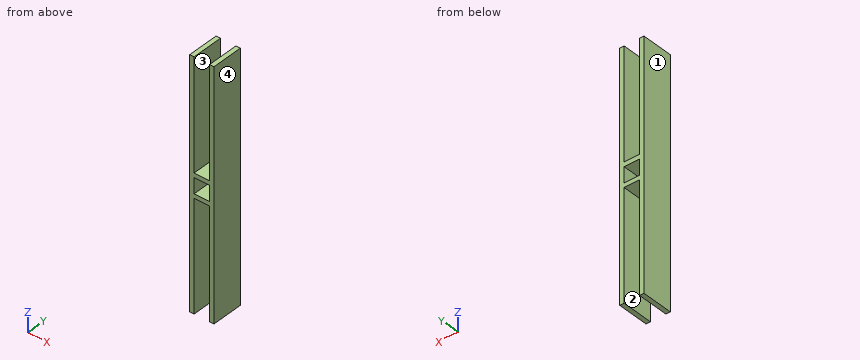
```python
from build123d import *

# Parameters (mm, degrees)
SKETCH1_W           = 10
SKETCH1_H           = 71
BOSS_EXTRUDE1_DEPTH = 556
SKETCH2_W           = 10
SKETCH2_H           = 71
BOSS_EXTRUDE2_DEPTH = 35
SKETCH3_W           = 10
SKETCH3_H           = 556
BOSS_EXTRUDE3_DEPTH = 71


with BuildPart() as part:
    # Sketch1 → Boss-Extrude1 (new body)
    with BuildSketch(Plane.XY):
        Rectangle(SKETCH1_W, SKETCH1_H)
    extrude(amount=BOSS_EXTRUDE1_DEPTH)

    # Sketch2 → Boss-Extrude2 (add)
    with BuildSketch(Plane(origin=(5, 0, 0), x_dir=(0, 0, -1), z_dir=(1, 0, 0))):
        with Locations((-300, 0)):
            Rectangle(SKETCH2_W, SKETCH2_H)
        with Locations((-255, 0)):
            Rectangle(SKETCH2_W, SKETCH2_H)
    extrude(amount=BOSS_EXTRUDE2_DEPTH)

    # Sketch3 → Boss-Extrude3 (add)
    with BuildSketch(Plane(origin=(0, 35.5, 0), x_dir=(1, 0, 0), z_dir=(0, 1, 0))):
        with Locations((45, -278)):
            Rectangle(SKETCH3_W, SKETCH3_H)
    extrude(amount=-BOSS_EXTRUDE3_DEPTH)


solid = part.part
```
The listing builds one solid part. Answer for the finished solid, in the listing's coordinates (mm). Face numbers are marked on the shaded views. Give positions to 0.01 mm unless a question says otherwise; leave off trailing zeros. Loops run counter-clockwise (first coordinate to the right, second up) from the corner with the lowest first, then second, coordinate; pieces in that order, holes last. Notation, with made-up numbers: (36.25, 73) - (44.25, 73) arc R25 ccw to (44.25, 86) - close; hole circle Ø1 at (31, 25). An arc over 180 degrees is marked (long way). Answer as CSV lines item,"result". Start each with the question number.
Item 1: Find the intervals of material crossed by line 1 (Z direction, x = 9, y = 13); line 2 (X direction, y = 23.5, z = 91.5), in increasing order. Write a range as from..to.
Item 2: This flat-tipped pin is pushed along its axis until it touches: pin 1 (4 mm diameter, centred on x = 39, z = 318.5, fed in from +Y). Where does it stop, or does it pass through?
Item 3: A cutting plane is placed at C-C on y = -27. Determine the outline of the cut face in (x, z), then the cut area to 3 significant figures.
Item 4: The mould has two halves that part along X. Classify the marked faces 1, 2, 3 and 4: +X half, -X half, draft (parallel to the pull), parting line (faces both ways), or undercut.
Item 5: A cutting plane is placed at B-B on x = 30. Determine the outline of the cut face in (y, z).
Item 6: A cutting plane is placed at A-A on z = 469.5. Determine the outline of the cut face in (x, y).
Found:
1,line 1,"z = 250..260, 295..305"
1,line 2,"x = -5..5, 40..50"
2,pin 1,"stops at y = 35.5"
3,outline,"(-5, 0) - (5, 0) - (5, 250) - (40, 250) - (40, 0) - (50, 0) - (50, 556) - (40, 556) - (40, 305) - (5, 305) - (5, 556) - (-5, 556) - close; hole (5, 260) - (40, 260) - (40, 295) - (5, 295) - close"
3,area,"11,800 mm^2"
4,face 1,"-X half"
4,face 2,"undercut"
4,face 3,"undercut"
4,face 4,"+X half"
5,outline,"(-35.5, 250) - (35.5, 250) - (35.5, 260) - (-35.5, 260) - close; (-35.5, 295) - (35.5, 295) - (35.5, 305) - (-35.5, 305) - close"
6,outline,"(-5, -35.5) - (5, -35.5) - (5, 35.5) - (-5, 35.5) - close; (40, -35.5) - (50, -35.5) - (50, 35.5) - (40, 35.5) - close"
